Read the model definition and answer for the solid it produces. Units are mm, in the model's axes. A direction names the side the tool comes from. Round coordinates to 2 decimals unless told otherwise and drop trailing zeros. Write each loop counter-clockwise with the first axis right and the second up, starting at its lowest first coordinate (ties: lowest second). Pieces come first, ordered by that corner, then holes.
from build123d import *

# Parameters (mm, degrees)
BOSS_EXTRUDE1_DEPTH     = 11.5
SKETCH2_OUTSIDE_W       = 75.842
SKETCH2_OUTSIDE_H       = 82.03
SKETCH2_OUTSIDE_R       = 20
CUT_EXTRUDE1_DEPTH      = 18
CUT_EXTRUDE1_DRAFT      = -30
MIRROR1_COPY_1_SKETCH_W = 75.842
MIRROR1_COPY_1_SKETCH_H = 82.03
MIRROR1_COPY_1_SKETCH_R = 20
MIRROR1_COPY_1_DEPTH    = 18
MIRROR1_COPY_1_DRAFT    = -30
SKETCH3_R               = 12.5
CUT_EXTRUDE2_DEPTH      = 18
SKETCH4_R               = 6
CUT_EXTRUDE3_DEPTH      = 18


with BuildPart() as part:
    # Sketch1 → Boss-Extrude1 (new, symmetric)
    with BuildSketch(Plane.XY):
        Polygon((0, 23.094010768), (-20, 11.547005384), (-20, -11.547005384), (0, -23.094010768), (20, -11.547005384), (20, 11.547005384), align=None)
    extrude(amount=BOSS_EXTRUDE1_DEPTH, both=True)


with BuildPart() as cut_extrude1_tool:
    # Sketch2 outside → Cut-Extrude1 (with draft: the straight prism first)
    with BuildSketch(Plane.XY.offset(11.5)):
        Rectangle(SKETCH2_OUTSIDE_W, SKETCH2_OUTSIDE_H)
        Circle(SKETCH2_OUTSIDE_R, mode=Mode.SUBTRACT)
    extrude(amount=-CUT_EXTRUDE1_DEPTH)
    # Cut-Extrude1: the draft: its side faces are tilted about the plane it starts from
    cut_extrude1_sides = [cut_extrude1_tool.faces().sort_by_distance(p)[0] for p in [
        (0, -41.015, 2.5),
        (37.921, 0, 2.5),
        (0, 41.015, 2.5),
        (-37.921, 0, 2.5),
        (-20, 0, 2.5),
    ]]
    draft(cut_extrude1_sides, Plane.XY.offset(11.5), CUT_EXTRUDE1_DRAFT)


with BuildPart() as part_1:
    add(part.part)

    # Cut-Extrude1: cut by cut_extrude1_tool
    add(cut_extrude1_tool.part, mode=Mode.SUBTRACT)


with BuildPart() as mirror1_copy_1_tool:
    # Mirror1 copy 1 sketch → Mirror1 copy 1 (with draft: the straight prism first)
    with BuildSketch(Plane(origin=(0, 0, -11.5), x_dir=(1, 0, 0), z_dir=(0, 0, -1))):
        Rectangle(MIRROR1_COPY_1_SKETCH_W, MIRROR1_COPY_1_SKETCH_H)
        Circle(MIRROR1_COPY_1_SKETCH_R, mode=Mode.SUBTRACT)
    extrude(amount=-MIRROR1_COPY_1_DEPTH)
    # Mirror1 copy 1: the draft: its side faces are tilted about the plane it starts from
    mirror1_copy_1_sides = [mirror1_copy_1_tool.faces().sort_by_distance(p)[0] for p in [
        (0, -41.015, -2.5),
        (37.921, 0, -2.5),
        (0, 41.015, -2.5),
        (-37.921, 0, -2.5),
        (-20, 0, -2.5),
    ]]
    draft(mirror1_copy_1_sides, Plane(origin=(0, 0, -11.5), x_dir=(1, 0, 0), z_dir=(0, 0, -1)), MIRROR1_COPY_1_DRAFT)


with BuildPart() as part_2:
    add(part_1.part)

    # Mirror1 copy 1: cut by mirror1_copy_1_tool
    add(mirror1_copy_1_tool.part, mode=Mode.SUBTRACT)

    # Sketch3 → Cut-Extrude2 (cut)
    with BuildSketch(Plane.XY.offset(11.5)):
        Circle(SKETCH3_R)
    extrude(amount=-CUT_EXTRUDE2_DEPTH, mode=Mode.SUBTRACT)

    # Sketch4 → Cut-Extrude3 (cut)
    with BuildSketch(Plane.XY.offset(-6.5)):
        Circle(SKETCH4_R)
    extrude(amount=-CUT_EXTRUDE3_DEPTH, mode=Mode.SUBTRACT)


solid = part_2.part
Q1. Flat-ended cylindrical pins translate along their axes: pin 1 Ø8 at (x, z) = (-7.5, -5) entering from +Y; pin 2 Ø1 at (x, y) = (12.5, -16.5) entering from +Z; pin 3 Ø2 at (x, z) = (-3, 3) entering from +Y. Find the tip coordinate at first contact, or state that the pin passes through.
Verdict:
pin 1: stops at y = 21.07
pin 2: passes through
pin 3: stops at y = 21.94
Q2. Straight lines are drawn through the part: probe 1 along Y at (x, z) = (0, -2.5); probe 2 along Z at (x, y) = (-10, 4.5); probe 3 along Y at (x, z) = (-8.5, 6.5). For each, find the intervals that lie inside material, in ascending order.
Verdict:
probe 1: y = -23.09 to -12.5, 12.5 to 23.09
probe 2: z = -11.5 to -6.5
probe 3: y = -18.19 to -9.17, 9.17 to 18.19
Q3. Section B-B (z = 7.25) is taken. Determine the outline of the cut face in (x, y), then the cut area to 3 significant figures.
Verdict:
outline: (-20, -10.21) arc R22.45 ccw to (-18.84, -12.22) - (-1.16, -22.42) arc R22.45 ccw to (1.16, -22.42) - (18.84, -12.22) arc R22.45 ccw to (20, -10.21) - (20, 10.21) arc R22.45 ccw to (18.84, 12.22) - (1.16, 22.42) arc R22.45 ccw to (-1.16, 22.42) - (-18.84, 12.22) arc R22.45 ccw to (-20, 10.21) - close; hole circle Ø25 at (0, 0)
area: 890 mm2
Q4. Determine the mould class of faces 1 (the flat face through (9, 9, 11.5)), 2 (the cylindrical face through (-6, 0, -9)), 3 (the cylindrical face through (11.923, 3.755, 2.626)), 4 (the conical face through (-0.05, -20.74, 10.22)) for opening direction Y: pulls with the +Y half, pulls with the -Y half, needs draft (parallel to the pull), parting line crosses it, or undercut.
Verdict:
face 1: needs draft
face 2: undercut
face 3: undercut
face 4: pulls with the -Y half
Q5. Section A-A (z = -3.75) is taken. Determine the outline of the cut face in (x, y), then the cut area to 3 significant figures.
Verdict:
outline: (-20, -11.55) - (0, -23.09) - (20, -11.55) - (20, 11.55) - (0, 23.09) - (-20, 11.55) - close; hole circle Ø25 at (0, 0)
area: 895 mm2
Q6. Which of the six approach directions +Z, -Z, +X, -X, +Y, -Y give full straight-line access (tool end or side, diameter ignored) to faces 5 (the flat face through (-3, -5.4, -6.5)), 6 (the conical face through (-17.934, -10.413, -10.222))?
Verdict:
face 5: +Z
face 6: -Z, -X, -Y
